Build history of the part. All positions in model axes, mm. Face numbers are marked on the shaded views. A direction names the side the tool comes from. Coordinates: 2 decimals unless noted, no trailing zeros. Loops run counter-clockwise (first coordinate to the right, second up) from the corner with the lowest first, then second, coordinate; pieces in that order, holes last.
Item 1: 3-axis set-ups, long thin cutter, end or side, ignore diameter. For the marked faces 1, 2 and 3: which of +Z, -Z, +X, -X, +Y, -Y reach the whole face in a straight line?
Item 2: Cut at C-C (x = -29). List the corners of the cut face in (y, z), and give its area (3 significant figures).
Item 3: Flat gauge pins, fed straight in: pin 1 (12 mm diameter, centred on x = -64.5, z = -121, fed in from -Y); pin 2 (1 mm diameter, centred on x = -46.5, z = -83.5, fed in from +Y); pin 3 (9 mm diameter, centred on x = -62.5, z = 56.25, fed in from -Y); pin 4 (3 mm diameter, centred on x = 60, z = 80, fed in from +Y). Where does each tip first touch, or does it go through?
Item 4: Cut at A-A (z = 0). List the corners of the cut face in (x, y).
Item 5: Cut at B-B (z = -65.5). List the corners of the cut face in (x, y), and give its area (3 significant figures).
Item 6: Drill centre lines: line 1 along X through (y, z) = (-3, 115); line 2 along Z through (x, y) = (50, -1.5); line 3 along Z through (x, y) = (57, -2.5). Where is each one in solid material? Low to high.
from build123d import *

# Parameters (mm, degrees)
SKETCH_1_W                   = 150
SKETCH_1_H                   = 330
EXTRUDE_1_DEPTH              = 10
SKETCH_2_W                   = 70
SKETCH_2_H                   = 330
CUT_EXTRUDE_1_DEPTH          = 3
SKETCH_3_W                   = 50
SKETCH_3_H                   = 330
CUT_EXTRUDE_2_DEPTH          = 8
MM_1_D                       = 1
HOLE_WIZARD_M6_1_D           = 6.6
HOLE_WIZARD_M6_1_CBORE_D     = 11
HOLE_WIZARD_M6_1_CBORE_DEPTH = 8
MM_0_D                       = 6
HOLE_WIZARD_M6_1_2_D         = 5
CHAMFER_1_SIZE               = 5
CUT_EXTRUDE_3_DEPTH          = 183.345825288
HOLE_WIZARD_M4_1_D           = 3.3


with BuildPart() as part:
    # 草图1 → 凸台-拉伸1 (new, symmetric)
    with BuildSketch(Plane(origin=(0, 0, 0), x_dir=(1, 0, 0), z_dir=(0, 1, 0))):
        Rectangle(SKETCH_1_W, SKETCH_1_H)
    extrude(amount=EXTRUDE_1_DEPTH, both=True)

    # 草图2 → 切除-拉伸1 (cut)
    with BuildSketch(Plane(origin=(0, 10, 0), x_dir=(1, 0, 0), z_dir=(0, 1, 0))):
        with Locations((-40, 0)):
            Rectangle(SKETCH_2_W, SKETCH_2_H)
    extrude(amount=-CUT_EXTRUDE_1_DEPTH, mode=Mode.SUBTRACT)

    # 草图3 → 切除-拉伸2 (cut)
    with BuildSketch(Plane(origin=(0, 10, 0), x_dir=(1, 0, 0), z_dir=(0, 1, 0))):
        with Locations((50, 0)):
            Rectangle(SKETCH_3_W, SKETCH_3_H)
    extrude(amount=-CUT_EXTRUDE_2_DEPTH, mode=Mode.SUBTRACT)

    # 大小mm 暗销孔1 (through all)
    with Locations(Plane(origin=(0, 7, 0), x_dir=(1, 0, 0), z_dir=(0, 1, 0))):
        with Locations((-62.500006208, 121.250006208), (-17.500006208, 121.250006208), (-62.500006208, 56.250006208), (-17.500006208, 56.250006208), (-62.500003219, -56.249995139), (-17.500003219, -56.249995139), (-62.500003219, -121.249995139), (-17.500003219, -121.249995139)):
            Hole(MM_1_D / 2)

    # Hole Wizard M6 _1 (through all)
    with Locations(Plane(origin=(0, -10, 0), x_dir=(-1, 0, 0), z_dir=(0, -1, 0))):
        with Locations((17.500006208, 121.250006208), (62.500006208, 121.250006208), (17.500006208, 56.250006208), (62.500006208, 56.250006208), (17.500003219, -56.249995139), (62.500003219, -56.249995139), (17.500003219, -121.249995139), (62.500003219, -121.249995139)):
            CounterBoreHole(HOLE_WIZARD_M6_1_D / 2, HOLE_WIZARD_M6_1_CBORE_D / 2, HOLE_WIZARD_M6_1_CBORE_DEPTH)

    # 大小mm 暗销孔0 (through all)
    with Locations(Plane(origin=(0, -10, 0), x_dir=(-1, 0, 0), z_dir=(0, -1, 0))):
        with Locations((-50.000000134, 114.999999999), (-50.000000032, -114.999999953), (49.999999866, 114.999999999), (49.999999968, -114.999999953)):
            Hole(MM_0_D / 2)

    # Hole Wizard M6 _1 2 (through all)
    with Locations(Plane(origin=(0, -10, 0), x_dir=(-1, 0, 0), z_dir=(0, -1, 0))):
        with Locations((59.999999968, -149.999999953), (-60.000000032, -149.999999953), (-60.000000032, -79.999999953), (59.999999968, -79.999999953), (59.999999866, 79.999999999), (59.999999866, 149.999999999), (-60.000000134, 149.999999999), (-60.000000134, 79.999999999)):
            Hole(HOLE_WIZARD_M6_1_2_D / 2)

    # 倒角1
    chamfer_1_edges = [part.edges().sort_by_distance(p)[0] for p in [
        (-75, -1.5, -165),
        (-75, -1.5, 165),
        (75, -4, -165),
        (75, -4, 165),
    ]]
    chamfer(chamfer_1_edges, length=CHAMFER_1_SIZE)

    # 草图14 → 切除-拉伸3 (cut, through all)
    with BuildSketch(Plane.XZ.offset(10)):
        with BuildLine():
            Line((50, 9.1), (60, 9.1))
            ThreePointArc((60, 9.1), (69.1, 0), (60, -9.1))
            Line((60, -9.1), (50, -9.1))
            ThreePointArc((50, -9.1), (40.9, 0), (50, 9.1))
        make_face()
    extrude(amount=-CUT_EXTRUDE_3_DEPTH, mode=Mode.SUBTRACT)

    # M4 螺纹孔1 (through all)
    with Locations(Plane(origin=(0, -10, 0), x_dir=(-1, 0, 0), z_dir=(0, -1, 0))):
        with Locations((-48.25000003, -35.000000224), (-48.25000003, -55.000000224), (48.249999938, -10.000000156), (48.249999938, 9.999999844)):
            Hole(HOLE_WIZARD_M4_1_D / 2)


solid = part.part
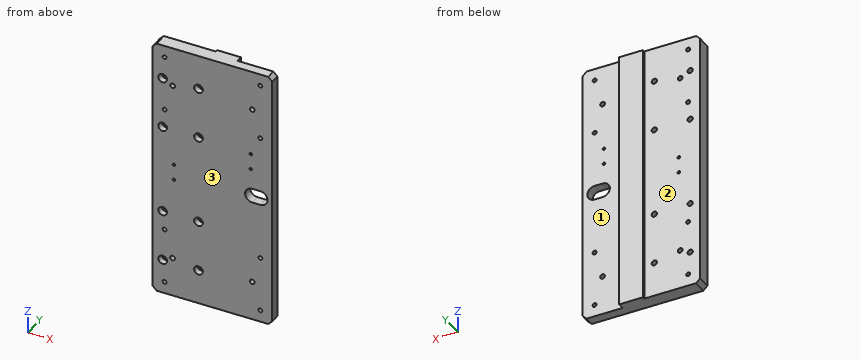
Filled sheet:
1. face 1: +Z, -Z, +X, +Y
1. face 2: +Z, -Z, -X, +Y
1. face 3: +Z, -Z, +X, -X, -Y
2. outline: (-10, -165) - (7, -165) - (7, 165) - (-10, 165) - close
2. area: 5,610 mm2
3. pin 1: stops at y = -10
3. pin 2: stops at y = 7
3. pin 3: stops at y = -2
3. pin 4: passes through
4. outline: (-75, -10) - (40.9, -10) - (40.9, 2) - (25, 2) - (25, 10) - (-5, 10) - (-5, 7) - (-75, 7) - close; (69.1, -10) - (75, -10) - (75, 2) - (69.1, 2) - close
5. outline: (-75, -10) - (75, -10) - (75, 2) - (25, 2) - (25, 10) - (-5, 10) - (-5, 7) - (-75, 7) - close
5. area: 2,390 mm2
6. line 1: x = -75 to -53, -47 to 47, 53 to 75
6. line 2: z = -165 to -118, -112 to -9.1, 9.1 to 112, 118 to 165
6. line 3: z = -165 to -9.1, 9.1 to 165
